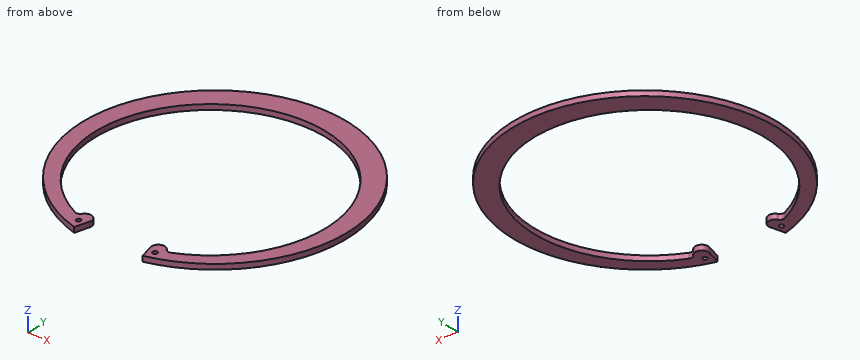
from build123d import *

# Parameters (mm, degrees)
SKETCH1_R          = 2
BASE_EXTRUDE_DEPTH = 2.375


with BuildPart() as part:
    # Sketch1 → Base-Extrude (new, symmetric)
    with BuildSketch(Plane.XY):
        with BuildLine():
            Line((-27.688947845, -103.336560167), (-31.122990174, -116.152580611))
            ThreePointArc((-31.122990174, -116.152580611), (0, 120.25), (31.122990174, -116.152580611))
            Line((31.122990174, -116.152580611), (27.688947845, -103.336560167))
            ThreePointArc((27.688947845, -103.336560167), (31.096993473, -96.279120559), (38.578543112, -98.613353586))
            ThreePointArc((38.578543112, -98.613353586), (40.821504489, -100.330026414), (43.639401714, -100.136903233))
            ThreePointArc((43.639401714, -100.136903233), (0, 100.05), (-43.639401714, -100.136903233))
            ThreePointArc((-43.639401714, -100.136903233), (-40.821504489, -100.330026414), (-38.578543112, -98.613353586))
            ThreePointArc((-38.578543112, -98.613353586), (-31.096993473, -96.279120559), (-27.688947845, -103.336560167))
        make_face()
        with Locations((-34.871256995, -106.959082997)):
            Circle(SKETCH1_R, mode=Mode.SUBTRACT)
        with Locations(Location((34.871256995, -106.959082997, 0), (0, 0, 180))):
            Circle(SKETCH1_R, mode=Mode.SUBTRACT)
    extrude(amount=BASE_EXTRUDE_DEPTH, both=True)


solid = part.part
Build history of the part. All positions in model axes, mm. Coordinates: 2 decimals unless noted, no trailing zeros. Write each loop counter-clockwise with the first axis right and the second up, starting at its lowest first coordinate (ties: lowest second). Pieces come first, ordered by that corner, then holes.
(1) Cut at C-C on z = 1.3. List the corners of the cut face in (x, y), and give its area (3 significant figures).
(2) Pin check, flat tips, straight feed: pin 1 Ø3 at (x, y) = (34.87, -106.96) entering from +Z; pin 2 Ø1.5 at (x, z) = (51, 2) entering from +Y. Stop position of each tip, or through.
(3) Drill centre lines: line 1 (X direction, y = 84, z = -0.25); line 2 (X direction, y = -4.8, z = -1.3); line 3 (Y direction, x = -85.5, z = -0.5). Where is each one in solid material? Low to high.
(4) Cut at A-A on x = 86.5. List the corners of the cut face in (y, z) (3 decimals).
(5) Cut at D-D on x = 0. List the corners of the cut face in (y, z) (3 decimals), and give its area (4 significant figures).
(6) Cut at B-B on y = 95.5. List the corners of the cut face in (x, z) (3 decimals), and give its area (3 significant figures).
Working result:
1. outline: (-43.64, -100.14) arc R104.85 cw (long way) to (43.64, -100.14) arc R4 cw to (38.58, -98.61) arc R6 ccw to (27.69, -103.34) - (31.12, -116.15) arc R120.25 ccw (long way) to (-31.12, -116.15) - (-27.69, -103.34) arc R6 ccw to (-38.58, -98.61) arc R4 cw to start; hole circle Ø4 at (-34.87, -106.96); hole circle Ø4 at (34.87, -106.96)
1. area: 10,400 mm2
2. pin 1: passes through
2. pin 2: stops at y = 109.25
3. line 1: x = -86.05 to -55.75, 55.75 to 86.05
3. line 2: x = -120.15 to -104.85, 104.85 to 120.15
3. line 3: y = -84.56 to -65.49, 55.89 to 84.56
4. outline: (-83.533, -2.375) - (-64.056, -2.375) - (-64.056, 2.375) - (-83.533, 2.375) - close; (54.456, -2.375) - (83.533, -2.375) - (83.533, 2.375) - (54.456, 2.375) - close
5. outline: (100.05, -2.375) - (120.25, -2.375) - (120.25, 2.375) - (100.05, 2.375) - close
5. area: 95.95 mm2
6. outline: (-73.074, -2.375) - (-30.552, -2.375) - (-30.552, 2.375) - (-73.074, 2.375) - close; (30.552, -2.375) - (73.074, -2.375) - (73.074, 2.375) - (30.552, 2.375) - close
6. area: 404 mm2
